The listing builds one solid part. Answer for the finished solid, in the listing's coordinates (mm). Face numbers are marked on the shaded views. A direction names the side the tool comes from. Give positions to 0.01 mm unless a question says otherwise; leave off trailing zeros. Write each loop counter-clockwise with the first axis right and the second up, starting at its lowest first coordinate (ties: lowest second). Pieces come first, ordered by that corner, then holes. Notation, with made-up numbers: (29, -31.5) -> (77, -31.5) arc R35 cw to (77, 6.5) -> close; hole circle Ø10 at (61, 51). An arc over 180 degrees is marked (long way). One line per question, with ' | ' between items.
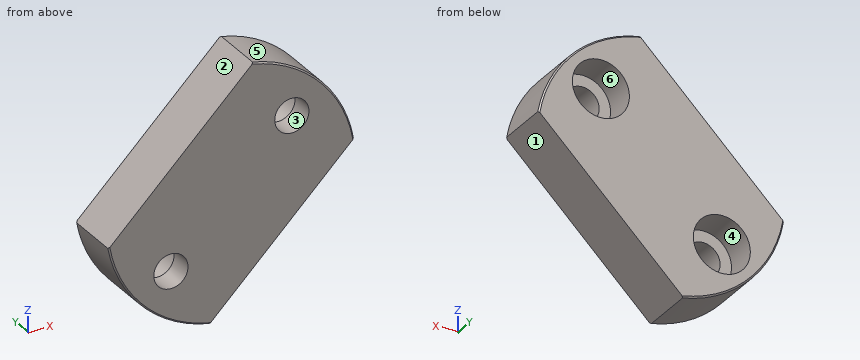
from build123d import *

# Parameters (mm, degrees)
G1_8_TAPPED_HOLE1_D                               = 8.8
HOLE_SIZE_BASED_ON_SOCKET_HEAD_CAP_SC_D           = 4.8
HOLE_SIZE_BASED_ON_SOCKET_HEAD_CAP_SC_CBORE_D     = 8
HOLE_SIZE_BASED_ON_SOCKET_HEAD_CAP_SC_CBORE_DEPTH = 4.6
FILLET1_R                                         = 0.2
CHAMFER1_SIZE                                     = 0.2
CHAMFER2_SIZE                                     = 0.5
CUT_EXTRUDE1_DEPTH                                = 35.474628352
SKETCH8_R                                         = 15
CUT_EXTRUDE2_DEPTH                                = 30.145808143
SKETCH9_R                                         = 7
BOSS_EXTRUDE1_DEPTH                               = 8


with BuildPart() as part:
    # Sketch2 → Revolve1 (revolve)
    with BuildSketch(Plane.XY, mode=Mode.PRIVATE) as revolve1_sk:
        Polygon((0, 24), (-17.5, 24), (-17.5, 16), (-6.75, 16), (-6.75, 0), (0, 0), align=None)
    revolve(revolve1_sk.sketch.rotate(Axis((0, 0, 0), (0, 1, 0)), 270), axis=Axis((0, 0, 0), (0, 1, 0)))

    # G1/8 Tapped Hole1 (through all)
    with Locations(Plane.ZX.offset(24)):
        with Locations((0, 0)):
            Hole(G1_8_TAPPED_HOLE1_D / 2)

    # Hole Size (% based on) Socket Head Cap Screw Type 1 (through all)
    with Locations(Plane(origin=(-8.485281374, 24, -8.485281374), x_dir=(0, 0, 1), z_dir=(0, 1, 0))):
        with Locations((0, 0), (16.970562748, 16.970562748)):
            CounterBoreHole(HOLE_SIZE_BASED_ON_SOCKET_HEAD_CAP_SC_D / 2, HOLE_SIZE_BASED_ON_SOCKET_HEAD_CAP_SC_CBORE_D / 2, HOLE_SIZE_BASED_ON_SOCKET_HEAD_CAP_SC_CBORE_DEPTH)

    # Fillet1
    fillet1_edges = [part.edges().sort_by_distance(p)[0] for p in [
        (0, 16, 6.75),
    ]]
    fillet(fillet1_edges, radius=FILLET1_R)

    # Chamfer1
    chamfer1_edges = [part.edges().sort_by_distance(p)[0] for p in [
        (0, 0, 6.75),
        (0, 16, 17.5),
        (0, 24, 17.5),
    ]]
    chamfer(chamfer1_edges, length=CHAMFER1_SIZE)

    # Chamfer2
    chamfer2_edges = [part.edges().sort_by_distance(p)[0] for p in [
        (0, 24, 4.4),
        (0, 0, 4.4),
    ]]
    chamfer(chamfer2_edges, length=CHAMFER2_SIZE)

    # Sketch7 → Cut-Extrude1 (cut, through all)
    with BuildSketch(Plane(origin=(0, 24, 0), x_dir=(1, 0, 0), z_dir=(0, 1, 0))):
        with BuildLine():
            Line((2.911166407, -17.053302031), (-17.053302031, 2.911166407))
            ThreePointArc((-17.053302031, 2.911166407), (-12.232947315, -12.232947315), (2.911166407, -17.053302031))
        make_face()
        with BuildLine():
            ThreePointArc((17.3, 0), (11.156317071, 13.222200627), (-2.911166407, 17.053302031))
            Line((-2.911166407, 17.053302031), (17.053302031, -2.911166407))
            ThreePointArc((17.053302031, -2.911166407), (17.238215179, -1.460800272), (17.3, 0))
        make_face()
        with BuildLine():
            Line((-17.053302031, 2.911166407), (-17.226115818, 3.083980194))
            ThreePointArc((-17.226115818, 3.083980194), (-12.374368671, -12.374368671), (3.083980194, -17.226115818))
            Line((3.083980194, -17.226115818), (2.911166407, -17.053302031))
            ThreePointArc((2.911166407, -17.053302031), (-12.232947315, -12.232947315), (-17.053302031, 2.911166407))
        make_face()
        with BuildLine():
            ThreePointArc((17.5, 0), (11.23121424, 13.42050024), (-3.083980194, 17.226115818))
            Line((-3.083980194, 17.226115818), (-2.911166407, 17.053302031))
            ThreePointArc((-2.911166407, 17.053302031), (11.156317071, 13.222200627), (17.3, 0))
            ThreePointArc((17.3, 0), (17.238215179, -1.460800272), (17.053302031, -2.911166407))
            Line((17.053302031, -2.911166407), (17.226115818, -3.083980194))
            ThreePointArc((17.226115818, -3.083980194), (17.431394477, -1.548058977), (17.5, 0))
        make_face()
    extrude(amount=-CUT_EXTRUDE1_DEPTH, mode=Mode.SUBTRACT)

    # Sketch8 → Cut-Extrude2 (cut, through all)
    with BuildSketch(Plane.XZ.offset(-16)):
        Circle(SKETCH8_R)
    extrude(amount=CUT_EXTRUDE2_DEPTH, mode=Mode.SUBTRACT)

    # Sketch9 → Boss-Extrude1 (add)
    with BuildSketch(Plane.XZ.offset(-16)):
        Circle(SKETCH9_R)
    extrude(amount=-BOSS_EXTRUDE1_DEPTH)


solid = part.part
Item 1: Consider line 1 (Z direction, x = 7, y = 19.5); line 2 (Z direction, x = -11, y = 23.5); line 3 (X direction, y = 20, z = 11). Determine where each line is inside the solid, lowest interval first. Write a range as [from, to].
Answers below:
line 1: [-7.14, 4.77], [12.2, 16.04] | line 2: [-13.61, -11.6], [-5.37, 3.14] | line 3: [-3.14, 5.37], [11.6, 13.61]
Item 2: Determine the mould class of the marked faces 1, 2, 3 and 4 for opening direction Z: pulls with the +Z half, pulls with the -Z half, needs draft (parallel to the pull), parting line crosses it, or undercut.
Answers below:
face 1: pulls with the -Z half | face 2: pulls with the +Z half | face 3: undercut | face 4: undercut
Item 3: Flat-ended cylindrical pins translate along their axes: pin 1 (9 mm diameter, centred on x = 8.49, z = 8.49, fed in from -Y); pin 2 (1 mm diameter, centred on x = 4.5, y = 18, fed in from +Z); pin 3 (3 mm diameter, centred on y = 20.5, z = -8.5, fed in from -X); pin 4 (1 mm diameter, centred on x = 0, y = 22, fed in from -Z). Find the tip coordinate at first contact, or state that the pin passes through.
Answers below:
pin 1: y = 16 | pin 2: z = 17.04 | pin 3: x = -16.04 | pin 4: z = -14.64
Item 4: Find section B-B (x = -1.5). Write down the section's boundary in (y, z).
Answers below:
outline: (16, -15.64) -> (24, -15.64) -> (24, 12.64) -> (16, 12.64) -> close
Item 5: Find section A-A (y = 16.75). Write down the section's boundary in (x, z).
Answers below:
outline: (-17.23, -3.08) arc R17.5 ccw to (-3.08, -17.23) -> (17.23, 3.08) arc R17.5 ccw to (3.08, 17.23) -> close; hole circle Ø4.8 at (-8.49, -8.49); hole circle Ø4.8 at (8.49, 8.49)
Item 6: A tool of negligible diameter and unlimited length cuts with its end or side. For the marked faces 5 and 6, from which of +Z, -Z, +X, -X, +Y, -Y can it reach the whole face along a straight path? Write none if from no direction.
Answers below:
face 5: +Z, +X, +Y, -Y | face 6: +Y
Item 7: Find section C-C (y = 22). Write down the section's boundary in (x, z).
Answers below:
outline: (-17.23, -3.08) arc R17.5 ccw to (-3.08, -17.23) -> (17.23, 3.08) arc R17.5 ccw to (3.08, 17.23) -> close; hole circle Ø8 at (-8.49, -8.49); hole circle Ø8 at (8.49, 8.49)
